Build history of the part. All positions in model axes, mm. A direction names the side the tool comes from. Round coordinates to 2 decimals unless told otherwise and drop trailing zeros. Order: outer loops, then holes, each group sorted by start corner. A loop starts at its lowest first (then second) coordinate and runs counter-clockwise, first axis right, second up. Notation, with made-up numbers: (64.5, 8) -> (82.5, 8) arc R36 ccw to (82.5, 45) -> close; hole circle Ø3 at (78.5, 43.25). An arc over 180 degrees is marked (long way). Write item = value, one per line.
from build123d import *

# Parameters (mm, degrees)
EXTRUDE_THIN1_DEPTH = 1649
SKETCH5_W           = 22
SKETCH5_H           = 64
CUT_EXTRUDE2_DEPTH  = 41


with BuildPart() as part:
    # Sketch3 → Extrude-Thin1 (new body)
    with BuildSketch(Plane(origin=(0, 0, 0), x_dir=(1, 0, 0), z_dir=(0, 1, 0))):
        Polygon((0, 40), (0, 0), (425, 0), (425, 40), (405, 40), (405, 25), (404, 25), (404, 41), (426, 41), (426, -1), (-1, -1), (-1, 40), align=None)
    extrude(amount=EXTRUDE_THIN1_DEPTH)

    # Sketch5 → Cut-Extrude2 (cut)
    with BuildSketch(Plane(origin=(0, 0, -41), x_dir=(-1, 0, 0), z_dir=(0, 0, -1))):
        with Locations((-415, 32)):
            Rectangle(SKETCH5_W, SKETCH5_H)
    extrude(amount=-CUT_EXTRUDE2_DEPTH, mode=Mode.SUBTRACT)


solid = part.part
Q1. Probe probe 1 along X at (y, z) = (1235, -33.5); probe 2 along X at (y, z) = (1005.5, -5); probe 3 along Z at (x, y) = (383, 499). List the from-to ranges inside material, lowest first.
Check values:
probe_1 = -1 to 0, 404 to 405, 425 to 426
probe_2 = -1 to 0, 425 to 426
probe_3 = 0 to 1
Q2. Cut at C-C, the plane x = 304. List the corners of the cut face in (y, z), and give its area (3 significant figures).
Check values:
outline = (0, 0) -> (1649, 0) -> (1649, 1) -> (0, 1) -> close
area = 1,650 mm²
Q3. Which spindle directions (+Z, -Z, +X, -X, +Y, -Y) get a long thin tool onto all of the face, cutting with end or side? Do faces 4 (the face through (-1, 813, -19)), 5 (the face through (0, 813, -20)). Say none if no direction does.
Check values:
face_4 = +Z, -Z, -X, +Y, -Y
face_5 = -Z, +Y, -Y
Q4. Cut at B-B, the plane y = 365. List the corners of the cut face in (x, z), and give its area (3 significant figures).
Check values:
outline = (-1, -40) -> (0, -40) -> (0, 0) -> (425, 0) -> (425, -40) -> (405, -40) -> (405, -25) -> (404, -25) -> (404, -41) -> (426, -41) -> (426, 1) -> (-1, 1) -> close
area = 544 mm²
Q5. Cut at A-A, the plane z = -14.5. List the corners of the cut face in (x, y), and give its area (3 significant figures).
Check values:
outline = (-1, 0) -> (0, 0) -> (0, 1649) -> (-1, 1649) -> close; (425, 64) -> (426, 64) -> (426, 1649) -> (425, 1649) -> close
area = 3,230 mm²
Q6. Flat gauge pins, fed straight in: pin 1 (8 mm diameter, centred on x = 269, y = 1067.5, fed in from -Z); pin 2 (24 mm diameter, centred on x = 416, z = -11, fed in from -Y); pin 3 (1.1 mm diameter, centred on x = -0.5, y = 833.5, fed in from -Z). Where does each tip first touch, or does it go through?
Check values:
pin_1 = 0
pin_2 = 0
pin_3 = -40
Q7. Mould opens along Z. For faces 1 (the face through (215, 813, 1)), 2 (the face through (426, 813, -20)), 3 (the face through (425, 845, -20)) say: released by +Z, released by -Z, zero draft, split by the parting line, or undercut.
Check values:
face_1 = released by +Z
face_2 = zero draft
face_3 = undercut
